from build123d import *

# Parameters (mm, degrees)
SKETCH1_R           = 32.5
SKETCH1_R_2         = 92.5
BOSS_EXTRUDE1_DEPTH = 40


with BuildPart() as part:
    # Sketch1 → Boss-Extrude1 (new body)
    with BuildSketch(Plane.XY):
        Polygon((240, 0), (-240, 0), (-255, 15), (-255, 90), (-587.5, 90), (-602.5, 105), (-602.5, 225), (-587.5, 240), (-407, 240), (-150, 365), (150, 365), (407, 240), (587.5, 240), (602.5, 225), (602.5, 105), (587.5, 90), (255, 90), (255, 15), align=None)
        with Locations((-200, 259)):
            Circle(SKETCH1_R, mode=Mode.SUBTRACT)
        with Locations(Location((200, 259, 0), (0, 0, 180))):
            Circle(SKETCH1_R, mode=Mode.SUBTRACT)
        with Locations((0, 242)):
            Circle(SKETCH1_R_2, mode=Mode.SUBTRACT)
    extrude(amount=BOSS_EXTRUDE1_DEPTH)


solid = part.part
Geometry: final body of the model. Coordinates: model frame, mm. A direction names the side the tool comes from. Round coordinates to 2 decimals unless told otherwise and drop trailing zeros. Loops run counter-clockwise (first coordinate to the right, second up) from the corner with the lowest first, then second, coordinate; pieces in that order, holes last. Notation, with made-up numbers: (46, 61.25) -> (54, 61.25) arc R8 ccw to (54, 71.25) -> close; hole circle Ø6 at (-34, 6). An arc over 180 degrees is marked (long way). One line per question, with ' | ' between items. Start each with the question number.
1. Section C-C on y = 208. Output: boundary loops of the cut face in (x, z).
2. Line query: line 1 along X through (y, z) = (284.5, 19.5); line 2 along Y through (x, z) = (481, 36); line 3 along X through (y, z) = (225, 33). Output: solid intervals per line, ascending. Write a range as [from, to].
3. Section D-D on y = 259. Output: boundary loops of the cut face in (x, z).
4. Set-up query: faces 1 (the face through (-499, 240, 20)), 2 (the face through (-255, 52, 20)), 3 (the face through (424, 90, 20)), 4 (the face through (496, 240, 20)). Return all of +Z, -Z, +X, -X, +Y, -Y with unobstructed straight access to the full face (end or side cutting, diameter ignored); none if empty.
5. Mould query, pull axis Y, two halves, no side actions, for faces 5 (the face through (42.683, 159.937, 19.72)), 6 (the face through (-280.299, 301.625, 19.72)), 7 (the face through (-419, 90, 20)). Classes: pulls with the +Y half, pulls with the -Y half, needs draft (parallel to the pull), parting line crosses it, or undercut.
6. Contact query for flat-ended pins moving along their axis: pin 1 (5 mm diameter, centred on x = 265.5, z = 33.5, fed in from -Y); pin 2 (4 mm diameter, centred on y = 283, z = 10, fed in from -X); pin 3 (1 mm diameter, centred on x = 247.5, y = 51.5, fed in from -Z); pin 4 (2 mm diameter, centred on y = 95, z = 30.5, fed in from -X). Output: stop coordinate, or through.
7. Section A-A on z = 13. Output: boundary loops of the cut face in (x, y).
8. Section B-B on x = 0. Output: boundary loops of the cut face in (y, z), and give its area (3 significant figures).
Returned:
1) outline: (-602.5, 0) -> (-86.02, 0) -> (-86.02, 40) -> (-602.5, 40) -> close; (86.02, 0) -> (602.5, 0) -> (602.5, 40) -> (86.02, 40) -> close
2) line 1: x = [-315.51, -220.15], [-179.85, -82.16], [82.16, 179.85], [220.15, 315.51] | line 2: y = [90, 240] | line 3: x = [-602.5, -90.92], [90.92, 602.5]
3) outline: (-367.94, 0) -> (-232.5, 0) -> (-232.5, 40) -> (-367.94, 40) -> close; (-167.5, 0) -> (-90.92, 0) -> (-90.92, 40) -> (-167.5, 40) -> close; (90.92, 0) -> (167.5, 0) -> (167.5, 40) -> (90.92, 40) -> close; (232.5, 0) -> (367.94, 0) -> (367.94, 40) -> (232.5, 40) -> close
4) face 1: +Z, -Z, -X, +Y | face 2: +Z, -Z, -X, -Y | face 3: +Z, -Z, +X, -Y | face 4: +Z, -Z, +X, +Y
5) face 5: undercut | face 6: pulls with the +Y half | face 7: pulls with the -Y half
6) pin 1: stops at y = 90 | pin 2: stops at x = -322.7 | pin 3: stops at z = 0 | pin 4: stops at x = -593.5
7) outline: (-602.5, 105) -> (-587.5, 90) -> (-255, 90) -> (-255, 15) -> (-240, 0) -> (240, 0) -> (255, 15) -> (255, 90) -> (587.5, 90) -> (602.5, 105) -> (602.5, 225) -> (587.5, 240) -> (407, 240) -> (150, 365) -> (-150, 365) -> (-407, 240) -> (-587.5, 240) -> (-602.5, 225) -> close; hole circle Ø65 at (-200, 259); hole circle Ø185 at (0, 242); hole circle Ø65 at (200, 259)
8) outline: (0, 0) -> (149.5, 0) -> (149.5, 40) -> (0, 40) -> close; (334.5, 0) -> (365, 0) -> (365, 40) -> (334.5, 40) -> close | area: 7,200 mm2
